Read the model definition and answer for the solid it produces. Units are mm, in the model's axes. Face numbers are marked on the shaded views. A direction names the side the tool comes from. Coordinates: 2 decimals unless noted, no trailing zeros. Loops run counter-clockwise (first coordinate to the right, second up) from the corner with the lowest first, then second, coordinate; pieces in that order, holes last. Notation, with made-up numbers: (73.5, 57) -> (114.5, 57) arc R22 cw to (114.5, 66) -> close; hole circle Ø5 at (66.25, 82.25). An arc over 180 degrees is marked (long way). Answer in a Markdown table with one row per item.
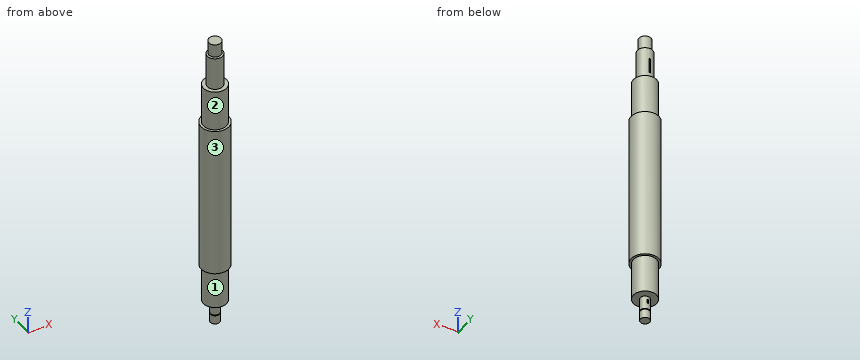
```python
from build123d import *

# Parameters (mm, degrees)
SKETCH1_R           = 15
BOSS_EXTRUDE1_DEPTH = 50
SKETCH2_R           = 18
BOSS_EXTRUDE2_DEPTH = 200
SKETCH3_R           = 15
BOSS_EXTRUDE3_DEPTH = 53
SKETCH4_R           = 6
BOSS_EXTRUDE4_DEPTH = 30
CUT_EXTRUDE1_START  = 5
CUT_EXTRUDE1_DEPTH  = 10
CUT_EXTRUDE3_START  = -12.5
SKETCH6_R           = 6
SKETCH6_R_2         = 5
CUT_EXTRUDE3_DEPTH  = 1
SKETCH7_R           = 10
BOSS_EXTRUDE5_DEPTH = 43
CUT_EXTRUDE4_START  = 4
CUT_EXTRUDE4_DEPTH  = 12
SKETCH8_R           = 8
BOSS_EXTRUDE6_DEPTH = 18
CUT_EXTRUDE6_START  = -18
SKETCH10_R          = 9
SKETCH10_R_2        = 7
CUT_EXTRUDE6_DEPTH  = 1


with BuildPart() as part:
    # Sketch1 → Boss-Extrude1 (new body)
    with BuildSketch(Plane.XY):
        Circle(SKETCH1_R)
    extrude(amount=BOSS_EXTRUDE1_DEPTH)

    # Sketch2 → Boss-Extrude2 (add)
    with BuildSketch(Plane.XY.offset(50)):
        Circle(SKETCH2_R)
    extrude(amount=BOSS_EXTRUDE2_DEPTH)

    # Sketch3 → Boss-Extrude3 (add)
    with BuildSketch(Plane.XY.offset(250)):
        Circle(SKETCH3_R)
    extrude(amount=BOSS_EXTRUDE3_DEPTH)

    # Sketch4 → Boss-Extrude4 (add)
    with BuildSketch(Plane(origin=(0, 0, 0), x_dir=(-1, 0, 0), z_dir=(0, 0, -1))):
        with Locations(Location((0, 0, 0), (0, 0, 180))):
            Circle(SKETCH4_R)
    extrude(amount=BOSS_EXTRUDE4_DEPTH)

    # Sketch5 → Cut-Extrude1 (cut)
    with BuildSketch(Plane(origin=(0, 0, 0), x_dir=(1, 0, 0), z_dir=(0, 1, 0)).offset(CUT_EXTRUDE1_START)):
        with BuildLine():
            ThreePointArc((-1, 9), (0, 8), (1, 9))
            Line((1, 9), (-1, 9))
        make_face()
        with BuildLine():
            Line((-1, 9), (1, 9))
            ThreePointArc((1, 9), (0, 10), (-1, 9))
        make_face()
        with BuildLine():
            Line((1, 5), (1, 9))
            ThreePointArc((1, 9), (0, 8), (-1, 9))
            Line((-1, 9), (-1, 5))
            ThreePointArc((-1, 5), (0, 6), (1, 5))
        make_face()
        with BuildLine():
            ThreePointArc((-1, 5), (0, 4), (1, 5))
            Line((1, 5), (-1, 5))
        make_face()
        with BuildLine():
            Line((-1, 5), (1, 5))
            ThreePointArc((1, 5), (0, 6), (-1, 5))
        make_face()
    extrude(amount=CUT_EXTRUDE1_DEPTH, mode=Mode.SUBTRACT)

    # Sketch6 → Cut-Extrude3 (cut)
    with BuildSketch(Plane(origin=(0, 0, -30), x_dir=(-1, 0, 0), z_dir=(0, 0, -1)).offset(CUT_EXTRUDE3_START)):
        with Locations(Location((0, 0, 0), (0, 0, 180))):
            Circle(SKETCH6_R)
        Circle(SKETCH6_R_2, mode=Mode.SUBTRACT)
    extrude(amount=CUT_EXTRUDE3_DEPTH, mode=Mode.SUBTRACT)

    # Sketch7 → Boss-Extrude5 (add)
    with BuildSketch(Plane.XY.offset(303)):
        Circle(SKETCH7_R)
    extrude(amount=BOSS_EXTRUDE5_DEPTH)

    # Sketch9 → Cut-Extrude4 (cut)
    with BuildSketch(Plane(origin=(0, 5, 0), x_dir=(1, 0, 0), z_dir=(0, 1, 0)).offset(CUT_EXTRUDE4_START)):
        with BuildLine():
            ThreePointArc((1, -313), (0, -314), (-1, -313))
            Line((-1, -313), (-1, -331))
            ThreePointArc((-1, -331), (0, -330), (1, -331))
            Line((1, -331), (1, -313))
        make_face()
        with BuildLine():
            ThreePointArc((1, -331), (0, -330), (-1, -331))
            Line((-1, -331), (1, -331))
        make_face()
        with BuildLine():
            Line((1, -331), (-1, -331))
            ThreePointArc((-1, -331), (0, -332), (1, -331))
        make_face()
        with BuildLine():
            ThreePointArc((1, -313), (0, -312), (-1, -313))
            Line((-1, -313), (1, -313))
        make_face()
        with BuildLine():
            Line((1, -313), (-1, -313))
            ThreePointArc((-1, -313), (0, -314), (1, -313))
        make_face()
    extrude(amount=CUT_EXTRUDE4_DEPTH, mode=Mode.SUBTRACT)

    # Sketch8 → Boss-Extrude6 (add)
    with BuildSketch(Plane.XY.offset(346)):
        Circle(SKETCH8_R)
    extrude(amount=BOSS_EXTRUDE6_DEPTH)

    # Sketch10 → Cut-Extrude6 (cut)
    with BuildSketch(Plane.XY.offset(364).offset(CUT_EXTRUDE6_START)):
        Circle(SKETCH10_R)
        Circle(SKETCH10_R_2, mode=Mode.SUBTRACT)
    extrude(amount=CUT_EXTRUDE6_DEPTH, mode=Mode.SUBTRACT)


solid = part.part
```
1. A cutting plane is placed at A-A on z = 258. Give the vertices of the cut face in (x, y).
A:
| item | result |
|---|---|
| outline | circle Ø30 at (0, 0) |
2. Find the intervals of material crossed by probe 1 along Z at (x, y) = (1.5, -5.5); probe 2 along Z at (x, y) = (-9.5, 3.5); probe 3 along X at (y, z) = (12, 271.5), in increasing order.
A:
| item | result |
|---|---|
| probe 1 | z = -30 to -18.5, -17.5 to 364 |
| probe 2 | z = 0 to 303 |
| probe 3 | x = -9 to 9 |
3. A tool of negligible diameter and unlimited length cuts with its end or side. For the marked faces 1, 2 and 3, from which of +Z, -Z, +X, -X, +Y, -Y can it reach the whole face along a straight path? Write none if from no direction.
A:
| item | result |
|---|---|
| face 1 | -Z |
| face 2 | +Z |
| face 3 | +Z, -Z |
4. A cutting plane is placed at B-B on z = 197.5. Give the vertices of the cut face in (x, y), and give its area (3 significant figures).
A:
| item | result |
|---|---|
| outline | circle Ø36 at (0, 0) |
| area | 1,020 mm2 |
5. Given pin 1 Ø12 at (y, z) = (11, 277) entering from -X; pin 2 Ø6 at (x, z) = (-5.5, 236.5) entering from +Y; pin 3 Ø15 at (x, y) = (-5, 7) entering from +Z; pin 4 Ø5 at (y, z) = (-8.5, 32) entering from +X, each flat-ended and moving along its own axis, determine where each tip first touches the part or whether it passes through.
A:
| item | result |
|---|---|
| pin 1 | stops at x = -14.14 |
| pin 2 | stops at y = 17.83 |
| pin 3 | stops at z = 364 |
| pin 4 | stops at x = 13.75 |
